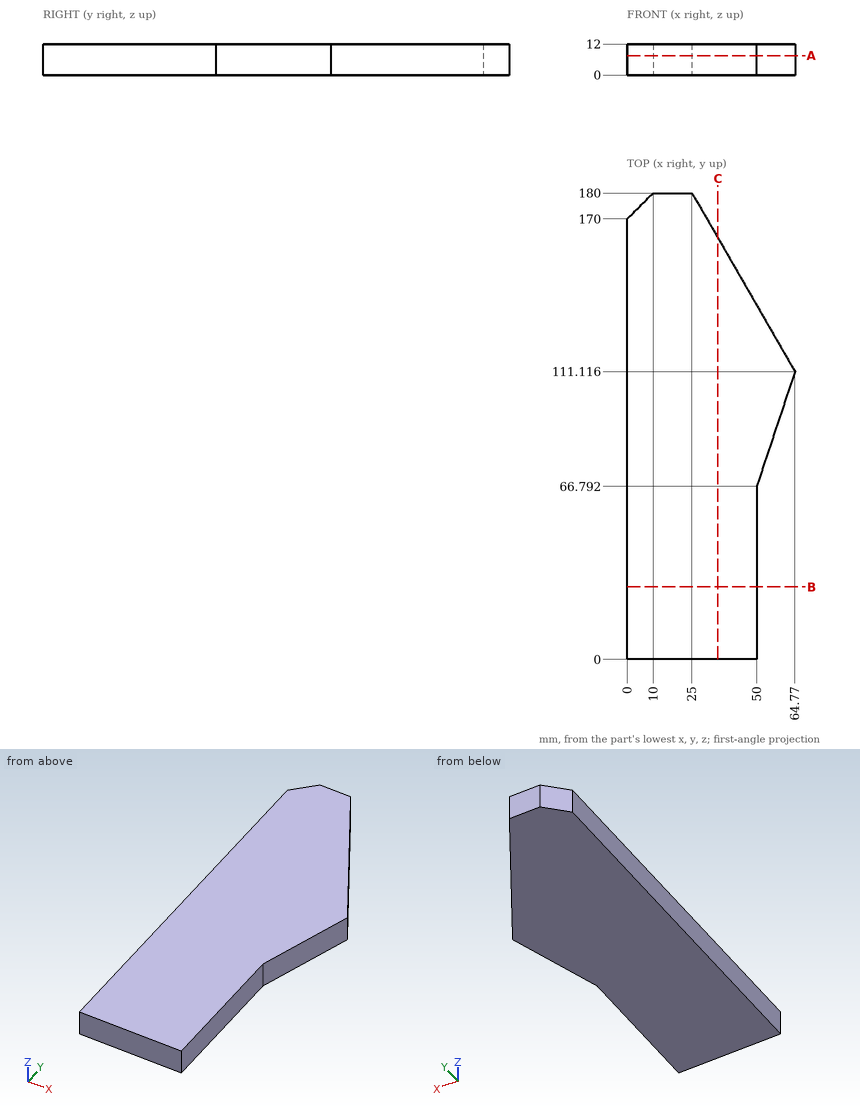
Study the drawing (mm; zero at the part's minimum x, y, z) and answer. Coordinates: 2 decimals unless noted, no trailing zeros. Order: outer loops, then holes, each group sorted by start corner. A loop starts at its lowest first (then second) coordinate and runs counter-clockwise, first axis right, second up. Notation, with made-up numbers: M -1.5,88 L 42.5,88 A24 cw 42.5,116 Z; hole C -10,10 d1. An arc over 180 degrees is marked long. Answer as a JSON object with one key per item and string values. Group by question number.
1. Straight lines are drawn through the part: line 1 (X direction, y = 33.5, z = 8); line 2 (X direction, y = 122.5, z = 2.75); line 3 (Y direction, x = 33, z = 5) (1 decimal). For each, find the intervals that lie inside material, in ascending order.
2. Flat-ended cylindrical pins translate along their axes: P1, Ø1, axis at y = 123.5, z = 5, coming from the +X side; P2, Ø4, axis at x = 37, y = 26.5, coming from the -Z side; P3, Ø3.5, axis at y = 49, z = 5, coming from the +X side. Find the tip coordinate at first contact, or state that the pin passes through.
3. Section B-B on y = 28 is taken. Write down the section's boundary in (x, z).
4. Section A-A on z = 7.5 is taken. Write down the section's boundary in (x, y), then the cut area to 4 significant figures.
5. Section C-C on x = 35 is taken. Write down the section's boundary in (y, z), then the cut area to 3 significant figures.
Values follow:
{
 "1": {"line 1": "0 to 50", "line 2": "0 to 58.2", "line 3": "0 to 166.1"},
 "2": {"P1": "x = 57.91", "P2": "z = 0", "P3": "x = 50"},
 "3": {"outline": "M 0,0 L 50,0 L 50,12 L 0,12 Z"},
 "4": {"outline": "M 0,0 L 50,0 L 50,66.79 L 64.77,111.12 L 25,180 L 10,180 L 0,170 Z", "area": "8,925 mm2"},
 "5": {"outline": "M 0,0 L 162.68,0 L 162.68,12 L 0,12 Z", "area": "1,950 mm2"}
}
